```python
from build123d import *

# Parameters (mm, degrees)
SKETCH_1_W                   = 120
SKETCH_1_H                   = 120
EXTRUDE_1_DEPTH              = 18
HOLE_WIZARD_M8_3_D           = 9
HOLE_WIZARD_M8_3_CBORE_D     = 15
HOLE_WIZARD_M8_3_CBORE_DEPTH = 10.6
SKETCH_11_W                  = 120
SKETCH_11_H                  = 74
CUT_EXTRUDE_2_DEPTH          = 2
CHAMFER_1_SIZE               = 5


with BuildPart() as part:
    # 草图1 → 凸台-拉伸1 (new body)
    with BuildSketch(Plane(origin=(0, 0, 0), x_dir=(1, 0, 0), z_dir=(0, 1, 0))):
        Rectangle(SKETCH_1_W, SKETCH_1_H)
    extrude(amount=EXTRUDE_1_DEPTH)

    # M8 六角凹头螺钉的柱形沉头孔3 (through all)
    with Locations(Plane(origin=(0, 18, 0), x_dir=(1, 0, 0), z_dir=(0, 1, 0))):
        with Locations((0, 40), (-34.641016151, 20), (-34.641016151, -20), (0, -40), (34.641016151, -20), (34.641016151, 20)):
            CounterBoreHole(HOLE_WIZARD_M8_3_D / 2, HOLE_WIZARD_M8_3_CBORE_D / 2, HOLE_WIZARD_M8_3_CBORE_DEPTH)

    # 草图11 → 切除-拉伸2 (cut)
    with BuildSketch(Plane(origin=(0, 18, 0), x_dir=(1, 0, 0), z_dir=(0, 1, 0))):
        Rectangle(SKETCH_11_W, SKETCH_11_H)
    extrude(amount=-CUT_EXTRUDE_2_DEPTH, mode=Mode.SUBTRACT)

    # 倒角1
    chamfer_1_edges = [part.edges().sort_by_distance(p)[0] for p in [
        (60, 9, 60),
        (-60, 9, 60),
        (-60, 9, -60),
        (60, 9, -60),
    ]]
    chamfer(chamfer_1_edges, length=CHAMFER_1_SIZE)


solid = part.part
```
Source: CAD feature listing. Evaluate the final solid. Frame: model axes, mm. A direction names the side the tool comes from. Coordinates: 2 decimals unless noted, no trailing zeros. Order: outer loops, then holes, each group sorted by start corner. A loop starts at its lowest first (then second) coordinate and runs counter-clockwise, first axis right, second up. Notation, with made-up numbers: M 32.5,60.25 L 66.5,60.25 A38 ccw 66.5,99.25 Z; hole C -23.75,79 d6. An arc over 180 degrees is marked long. Write each question's results on one line, items separated by ' | '. Start each with the question number.
1) Section query C-C (y = 12.75). Return the cut outline in (x, z), plus the area to 3 significant figures.
2) Contact query for flat-ended pins moving along their axis: pin 1 Ø14.5 at (x, z) = (34.64, -20) entering from +Y; pin 2 Ø17 at (x, z) = (-34.64, -20) entering from +Y; pin 3 Ø4.5 at (x, z) = (34.5, -19) entering from +Y. Output: stop coordinate, or through.
3) Draft query along Z for faces 1 (the face through (32.222, 3.648, -23.794)), 2 (the face through (60, 9, 1)), 3 (the face through (-1, 9, 60)). Return one class per face: released by +Z, released by -Z, zero draft, split by the parting line, or undercut.
4) Section query B-B (z = -20). Return the cut outline in (x, y), plus the area to 3 significant figures.
5) Access query for faces 4 (the face through (-1, 16, -1)), 5 (the face through (-1, 0, -1)), 6 (the face through (40, 7.4, -20)). Directions: +Z, -Z, +X, -X, +Y, -Y. A direction counts if a zero-diameter tool reaches every point of the face in a straight line with its end or side. Return the directions, or none.
6) Line query: line 1 (X direction, y = 4.25, z = 19.5); line 2 (Z direction, x = 0, y = 4); line 3 (Z direction, x = 0, y = 15.25). Output: solid intervals per line, ascending. Write a range as from..to.
7) Section query D-D (z = -40). Return the cut outline in (x, y), plus the area to 3 significant figures.
8) Section query A-A (x = 0). Return the cut outline in (y, z), plus the area to 3 significant figures.
Answers:
1) outline: M -60,-55 L -55,-60 L 55,-60 L 60,-55 L 60,55 L 55,60 L -55,60 L -60,55 Z; hole C -34.64,-20 d15; hole C -34.64,20 d15; hole C 0,-40 d15; hole C 0,40 d15; hole C 34.64,-20 d15; hole C 34.64,20 d15 | area: 13,300 mm^2
2) pin 1: stops at y = 7.4 | pin 2: stops at y = 16 | pin 3: passes through
3) face 1: undercut | face 2: zero draft | face 3: released by +Z
4) outline: M -60,0 L -39.14,0 L -39.14,7.4 L -42.14,7.4 L -42.14,16 L -60,16 Z; M -30.14,0 L 30.14,0 L 30.14,7.4 L 27.14,7.4 L 27.14,16 L -27.14,16 L -27.14,7.4 L -30.14,7.4 Z; M 39.14,0 L 60,0 L 60,16 L 42.14,16 L 42.14,7.4 L 39.14,7.4 Z | area: 1,530 mm^2
5) face 4: +X, -X, +Y | face 5: +Z, -Z, +X, -X, -Y | face 6: +Y
6) line 1: x = -60..-39.11, -30.17..30.17, 39.11..60 | line 2: z = -60..-44.5, -35.5..35.5, 44.5..60 | line 3: z = -60..-47.5, -32.5..32.5, 47.5..60
7) outline: M -60,0 L -4.5,0 L -4.5,7.4 L -7.5,7.4 L -7.5,18 L -60,18 Z; M 4.5,0 L 60,0 L 60,18 L 7.5,18 L 7.5,7.4 L 4.5,7.4 Z | area: 1,930 mm^2
8) outline: M 0,-60 L 18,-60 L 18,-47.5 L 7.4,-47.5 L 7.4,-44.5 L 0,-44.5 Z; M 0,-35.5 L 7.4,-35.5 L 7.4,-32.5 L 16,-32.5 L 16,32.5 L 7.4,32.5 L 7.4,35.5 L 0,35.5 Z; M 0,44.5 L 7.4,44.5 L 7.4,47.5 L 18,47.5 L 18,60 L 0,60 Z | area: 1,580 mm^2
